from build123d import *

# Parameters (mm, degrees)
SKETCH_1_W          = 308.5
SKETCH_1_H          = 220
EXTRUDE_1_DEPTH     = 30
SKETCH_2_W          = 366.462982974
SKETCH_2_H          = 68.169207718
CUT_EXTRUDE_1_DEPTH = 15


with BuildPart() as part:
    # 草图1 → 凸台-拉伸1 (new body)
    with BuildSketch(Plane(origin=(0, 0, 0), x_dir=(1, 0, 0), z_dir=(0, 1, 0))):
        Rectangle(SKETCH_1_W, SKETCH_1_H)
    extrude(amount=EXTRUDE_1_DEPTH)

    # 草图2 → 切除-拉伸1 (cut)
    with BuildSketch(Plane(origin=(0, 30, 0), x_dir=(1, 0, 0), z_dir=(0, 1, 0))):
        with Locations((15.777271283, 114.084603859)):
            Rectangle(SKETCH_2_W, SKETCH_2_H)
    extrude(amount=-CUT_EXTRUDE_1_DEPTH, mode=Mode.SUBTRACT)


solid = part.part
Source: CAD feature listing. Evaluate the final solid. Frame: model axes, mm. A direction names the side the tool comes from. Give positions to 0.01 mm unless a question says otherwise; leave off trailing zeros. Order: outer loops, then holes, each group sorted by start corner. A loop starts at its lowest first (then second) coordinate and runs counter-clockwise, first axis right, second up. Notation, with made-up numbers: (61.5, -29.5) -> (92.5, -29.5) arc R28 cw to (92.5, 2.5) -> close; hole circle Ø3 at (77, -22.75). An arc over 180 degrees is marked (long way). Use a Markdown table: item, result.
1) Section query C-C, the plane z = -92.5. Return the cut outline in (x, y).
Answer list:
| item | result |
|---|---|
| outline | (-154.25, 0) -> (154.25, 0) -> (154.25, 15) -> (-154.25, 15) -> close |
2) Section query A-A, the plane x = 55. Return the cut outline in (y, z).
Answer list:
| item | result |
|---|---|
| outline | (0, -110) -> (15, -110) -> (15, -80) -> (30, -80) -> (30, 110) -> (0, 110) -> close |
3) Contact query for a flat-ended pin moving along its axis: P1, Ø7.5, axis at x = -49, y = 20.5, coming from the -Z side. Output: stop coordinate, or through.
Answer list:
| item | result |
|---|---|
| P1 | z = -80 |
4) Ray query, line 1 along Z through (x, y) = (-21, 18); line 2 along Y through (x, z) = (100, -81.5). Return the intervals inside material, ascending. Write a range as [from, to].
Answer list:
| item | result |
|---|---|
| line 1 | [-80, 110] |
| line 2 | [0, 15] |
5) Section query B-B, the plane y = 24.25. Return the cut outline in (x, z), then the cut area to 3 significant figures.
Answer list:
| item | result |
|---|---|
| outline | (-154.25, -80) -> (154.25, -80) -> (154.25, 110) -> (-154.25, 110) -> close |
| area | 58,600 mm² |
6) Reachability of faces 1 (the flat face through (-154.25, 15, 2)), 2 (the flat face through (-2, 23, -80)) from +Z, -Z, +X, -X, +Y, -Y: full face, straight path, thin tool, end or side. Return the list, or none.
Answer list:
| item | result |
|---|---|
| face 1 | +Z, -Z, -X, +Y, -Y |
| face 2 | -Z, +X, -X, +Y |
